```python
from build123d import *

# Parameters (mm, degrees)
L_BLOCK_BASE_DEPTH      = 100
KEYED_BORE_CUT_DEPTH    = 50
STEP_BOSS_DEPTH         = 60
STEP_CUT_DEPTH          = 44
STEP_RELIEF_CUT_DEPTH   = 4
LOW_STEP_SLOT_CUT_DEPTH = 28


with BuildPart() as part:
    # L-Block Profile Sketch → L-Block Base (new body)
    with BuildSketch(Plane.XY):
        Polygon((0, 0), (150, 0), (150, 100), (94, 100), (94, 28), (0, 28), align=None)
    extrude(amount=L_BLOCK_BASE_DEPTH)

    # Keyed Bore Sketch → Keyed Bore Cut (cut)
    with BuildSketch(Plane(origin=(0, 100, 0), x_dir=(1, 0, 0), z_dir=(0, 1, 0))):
        with BuildLine():
            Line((113, -69.228756555), (131, -69.228756555))
            Line((131, -69.228756555), (131, -63.228756555))
            ThreePointArc((131, -63.228756555), (138, -50), (131, -36.771243445))
            Line((131, -36.771243445), (131, -30.771243445))
            Line((131, -30.771243445), (113, -30.771243445))
            Line((113, -30.771243445), (113, -36.771243445))
            ThreePointArc((113, -36.771243445), (106, -50), (113, -63.228756555))
            Line((113, -63.228756555), (113, -69.228756555))
        make_face()
    extrude(amount=-KEYED_BORE_CUT_DEPTH, mode=Mode.SUBTRACT)

    # Step Boss Sketch → Step Boss (add)
    with BuildSketch(Plane.XY.offset(100)):
        Polygon((94, 28), (94, 76), (56, 28), align=None)
    extrude(amount=-STEP_BOSS_DEPTH)

    # Step Cut Sketch → Step Cut (cut)
    with BuildSketch(Plane.XY.offset(100)):
        Polygon((94, 76), (94, 28), (56, 28), align=None)
    extrude(amount=-STEP_CUT_DEPTH, mode=Mode.SUBTRACT)

    # Step Relief Sketch → Step Relief Cut (cut)
    with BuildSketch(Plane(origin=(0, 0, 40), x_dir=(-1, 0, 0), z_dir=(0, 0, -1))):
        Polygon((-94, 76), (-94, 28), (-56, 28), align=None)
    extrude(amount=-STEP_RELIEF_CUT_DEPTH, mode=Mode.SUBTRACT)

    # Low Step Slot Sketch → Low Step Slot Cut (cut)
    with BuildSketch(Plane(origin=(0, 28, 0), x_dir=(1, 0, 0), z_dir=(0, 1, 0))):
        with BuildLine():
            Line((0, -34), (0, -66))
            Line((0, -66), (36, -66))
            ThreePointArc((36, -66), (52, -50), (36, -34))
            Line((36, -34), (0, -34))
        make_face()
    extrude(amount=-LOW_STEP_SLOT_CUT_DEPTH, mode=Mode.SUBTRACT)


solid = part.part
```
Verification items for the finished model (mm, model axes). A direction names the side the tool comes from. Coordinates: 2 decimals unless noted, no trailing zeros. Loops run counter-clockwise (first coordinate to the right, second up) from the corner with the lowest first, then second, coordinate; pieces in that order, holes last. Notation, with made-up numbers: (32.5, -9.5) -> (50.5, -9.5) arc R31 ccw to (50.5, 27.5) -> close; hole circle Ø1 at (8.5, 29). An arc over 180 degrees is marked (long way). Put each result on its own line as item: value.
1. Section check D-D, the plane z = 50. Record the boundary of the cut face in (x, y).
Result set:
outline: (52, 0) -> (150, 0) -> (150, 100) -> (138, 100) -> (138, 50) -> (106, 50) -> (106, 100) -> (94, 100) -> (94, 76) -> (56, 28) -> (52, 28) -> close
2. Section check B-B, the plane x = 119. Record the boundary of the cut face in (y, z).
Result set:
outline: (0, 0) -> (100, 0) -> (100, 30.77) -> (50, 30.77) -> (50, 69.23) -> (100, 69.23) -> (100, 100) -> (0, 100) -> close
3. Section check A-A, the plane y = 60. Record the boundary of the cut face in (x, z).
Result set:
outline: (81.33, 44) -> (94, 44) -> (94, 0) -> (150, 0) -> (150, 100) -> (94, 100) -> (94, 56) -> (81.33, 56) -> close; hole (113, 30.77) -> (131, 30.77) -> (131, 36.77) arc R16 ccw to (131, 63.23) -> (131, 69.23) -> (113, 69.23) -> (113, 63.23) arc R16 ccw to (113, 36.77) -> close
4. Tool access check on faces 4 (the face through (48, 28, 38)), 5 (the face through (18, 14, 34)), 6 (the face through (113, 75, 34)), 7 (the face through (107, 40, 0)). Record the directions out of +Z, -Z, +X, -X, +Y, -Y that give a thin tool (end or side, any length) a straight path to the whole face; none if there is none.
Result set:
face 4: -X, +Y
face 5: -X, +Y, -Y
face 6: +Y
face 7: -Z, +X, -X, +Y, -Y
5. Gauge pin test, flat ends, axial feed: P1, Ø6.5, axis at y = 83, z = 66.5, coming from the -X side; P2, Ø16, axis at x = 124, z = 41.5, coming from the +Y side; P3, Ø11.5, axis at x = 81, y = 46, coming from the -Z side; P4, Ø14.5, axis at x = 124.5, y = 75.5, coming from the -Z side. Record the tip position at first contact, or that the pin passes through.
Result set:
P1: stops at x = 94
P2: stops at y = 50
P3: stops at z = 44
P4: stops at z = 0
6. Section check C-C, the plane z = 83.5. Record the boundary of the cut face in (x, y), then the cut area to 3 significant figures.
Result set:
outline: (0, 0) -> (150, 0) -> (150, 100) -> (94, 100) -> (94, 28) -> (0, 28) -> close
area: 8,230 mm^2
7. Thickness scan on line 1 (X direction, y = 41, z = 94.5); line 2 (Y direction, x = 71.5, z = 92.5); line 3 (X direction, y = 92, z = 52). Record the ranges inside material, lowest first.
Result set:
line 1: x = 94 to 150
line 2: y = 0 to 28
line 3: x = 94 to 106.13, 137.87 to 150
8. Mould release check, pull along Z, two halves, no side actions. Record for faces 1 (the face through (84, 42, 44)), 2 (the face through (122, 75, 69.229)), 3 (the face through (0, 14, 83)): pulls with the +Z half, pulls with the -Z half, needs draft (parallel to the pull), parting line crosses it, or undercut.
Result set:
face 1: pulls with the -Z half
face 2: undercut
face 3: needs draft
